The model under review builds one solid part; all positions refer to its coordinate system, in mm. Face numbers are marked on the shaded views. Give positions to 0.01 mm unless a question says otherwise; leave off trailing zeros. Order: outer loops, then holes, each group sorted by start corner. A loop starts at its lowest first (then second) coordinate and runs counter-clockwise, first axis right, second up.
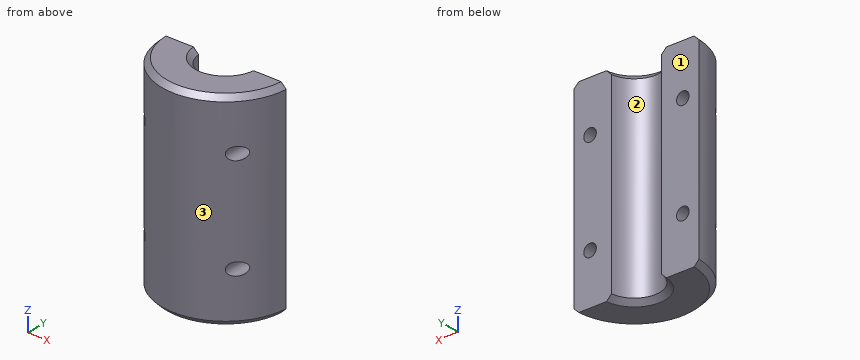
```python
from build123d import *

# Parameters (mm, degrees)
EXTRUDE_1_DEPTH    = 80
HOLE_WIZARD_M6_1_D = 5
CHAMFER_1_SIZE     = 2


with BuildPart() as part:
    # 草图1 → 凸台-拉伸1 (new body)
    with BuildSketch(Plane.XY):
        with BuildLine():
            Line((-24.979991994, -1), (-9.949874371, -1))
            ThreePointArc((-9.949874371, -1), (0, -10), (9.949874371, -1))
            Line((9.949874371, -1), (24.979991994, -1))
            ThreePointArc((24.979991994, -1), (0, -25), (-24.979991994, -1))
        make_face()
    extrude(amount=EXTRUDE_1_DEPTH)

    # M6 螺纹孔1 (through all)
    with Locations(Plane(origin=(0, -1, 0), x_dir=(1, 0, 0), z_dir=(0, 1, 0))):
        with Locations((-18.5, -20), (18.5, -20), (18.5, -60), (-18.5, -60)):
            Hole(HOLE_WIZARD_M6_1_D / 2)

    # 倒角1
    chamfer_1_edges = [part.edges().sort_by_distance(p)[0] for p in [
        (0, -25, 80),
        (0, -10, 80),
        (0, -25, 0),
        (0, -10, 0),
    ]]
    chamfer(chamfer_1_edges, length=CHAMFER_1_SIZE)


solid = part.part
```
1. Insertion check: pin 1 (2 mm diameter, centred on y = -13, z = 39, fed in from -X); pin 2 (5 mm diameter, centred on y = -16, z = 27, fed in from +X); pin 3 (4 mm diameter, centred on x = -6, z = 28.5, fed in from +Y). Each pin has a flat end and moves straight along its axis. Give the tip position at first contact, or say it passes through.
2. Draft analysis for pull direction X (two halves, no side actions). For the marked faces 1, 2 and 3, state which applies: pulls with the +X half, pulls with the -X half, needs draft (parallel to the pull), parting line crosses it, or undercut.
3. To check wall thickness, follow line 1 (Z direction, x = -18.5, y = -12.5); line 2 (X direction, y = -5, z = 20); line 3 (X direction, y = -7, z = 60). State the ranges of each line that lie inside material, in increasing order.
4. Take a section at A-A (x = 0). Write out the cut boundary in (y, z), and give its area (3 significant figures).
5. Take a section at B-B (z = 60). Write out the cut boundary in (x, y).
6. Take a section at C-C (y = -8.5). Count the separate pieces of the cut face and the enclosed holes in it, and give its area (3 significant figures).
Answer:
1. pin 1: stops at x = -21.93
1. pin 2: stops at x = 21.04
1. pin 3: stops at y = -6
2. face 1: needs draft
2. face 2: undercut
2. face 3: parting line crosses it
3. line 1: z = 0 to 17.5, 22.5 to 57.5, 62.5 to 80
3. line 2: x = -24.49 to -21, -16 to -8.66, 8.66 to 16, 21 to 24.49
3. line 3: x = -24 to -21, -16 to -7.14, 7.14 to 16, 21 to 24
4. outline: (-25, 2) - (-23, 0) - (-12, 0) - (-10, 2) - (-10, 78) - (-12, 80) - (-23, 80) - (-25, 78) - close
4. area: 1,190 mm2
5. outline: (-24.98, -1) arc R25 ccw to (-21, -13.56) - (-21, -1) - close; (-16, -19.21) arc R25 ccw to (16, -19.21) - (16, -1) - (9.95, -1) arc R10 cw to (-9.95, -1) - (-16, -1) - close; (21, -13.56) arc R25 ccw to (24.98, -1) - (21, -1) - close
6. separate pieces: 2
6. enclosed holes: 4
6. area: 2,820 mm2
